```python
from build123d import *

# Parameters (mm, degrees)
SKETCH1_R           = 8
BOSS_EXTRUDE1_DEPTH = 16
FILLET1_R           = 2
FILLET2_R           = 2


with BuildPart() as part:
    # Sketch1 → Boss-Extrude1 (new body)
    with BuildSketch(Plane(origin=(0, 0, 0), x_dir=(1, 0, 0), z_dir=(0, 1, 0))):
        Polygon((5.636967427, -10.593611199), (11.992820129, -0.415048607), (6.355852702, 10.178562591), (-5.636967427, 10.593611199), (-11.992820129, 0.415048607), (-6.355852702, -10.178562591), align=None)
        with Locations(Location((0, 0, 0), (0, 0, 270))):
            Circle(SKETCH1_R, mode=Mode.SUBTRACT)
    extrude(amount=BOSS_EXTRUDE1_DEPTH)

    # Fillet1
    fillet1_edges = [part.edges().sort_by_distance(p)[0] for p in [
        (5.636967427, 8, 10.593611199),
    ]]
    fillet(fillet1_edges, radius=FILLET1_R)

    # Fillet2
    fillet2_edges = [part.edges().sort_by_distance(p)[0] for p in [
        (-6.355852702, 8, 10.178562591),
        (-11.992820129, 8, -0.415048607),
        (-5.636967427, 8, -10.593611199),
        (6.355852702, 8, -10.178562591),
        (11.992820129, 8, 0.415048607),
    ]]
    fillet(fillet2_edges, radius=FILLET2_R)


solid = part.part
```
Geometry check sheet. Reference: the model listing, model coordinates, mm. Give positions to 0.01 mm unless a question says otherwise; leave off trailing zeros. Order: outer loops, then holes, each group sorted by start corner. A loop starts at its lowest first (then second) coordinate and runs counter-clockwise, first axis right, second up.
1. Section check B-B, the plane z = 2.75. Enter the section's corners in (x, y), and give its area (3 significant figures).
2. Section check D-D, the plane z = -8.5. Enter the section's corners in (x, y), and give its area (3 significant figures).
3. Section check C-C, the plane x = 0. Enter the section's corners in (y, z).
4. Release check for a two-part mould opening along Z. For faces 1 (the face through (6.2, 8.11, -9.91)), 2 (the face through (8.78, 7.89, 5.56)), 3 (the face through (-7.81, 7.89, -1.73)) record: pulls with the +Z half, pulls with the -Z half, needs draft (parallel to the pull), parting line crosses it, or undercut.
5. Gauge pin test, flat ends, axial feed: pin 1 Ø1 at (x, z) = (-9, 3) entering from -Y; pin 2 Ø6 at (y, z) = (2, 7.5) entering from -X; pin 3 Ø4 at (x, z) = (0, -4) entering from -Y; pin 4 Ø5 at (x, y) = (-1, 3.5) entering from -Z. Record the tip position at first contact, or that the pin passes through.
6. Section check A-A, the plane y = 4.75. Enter the section's corners in (x, z), and give its area (3 significant figures).
7. Thickness scan on L1, parallel to X at y = 10.5, z = 0; L2, parallel to Z at x = 2, y = 2.75; L3, parallel to X at y = 11.75, z = 2. Record the ranges inside material, lowest first.
Values follow:
1. outline: (-10.31, 0) - (-7.51, 0) - (-7.51, 16) - (-10.31, 16) - close; (7.51, 0) - (10.53, 0) - (10.53, 16) - (7.51, 16) - close
1. area: 93.1 mm2
2. outline: (-6.94, 0) - (7.25, 0) - (7.25, 16) - (-6.94, 16) - close
2. area: 227 mm2
3. outline: (0, -10.4) - (16, -10.4) - (16, -8) - (0, -8) - close; (0, 8) - (16, 8) - (16, 10.4) - (0, 10.4) - close
4. face 1: pulls with the -Z half
4. face 2: pulls with the +Z half
4. face 3: undercut
5. pin 1: stops at y = 0
5. pin 2: stops at x = -9.38
5. pin 3: passes through
5. pin 4: stops at z = -10.52
6. outline: (-11.45, 0.6) arc R2 ccw to (-11.38, -1.39) - (-6.25, -9.61) arc R2 ccw to (-4.48, -10.55) - (5.2, -10.22) arc R2 ccw to (6.9, -9.16) - (11.45, -0.6) arc R2 ccw to (11.38, 1.39) - (6.25, 9.61) arc R2 ccw to (4.48, 10.55) - (-5.2, 10.22) arc R2 ccw to (-6.9, 9.16) - close; hole circle Ø16 at (0, 0)
6. area: 172 mm2
7. L1: x = -11.66 to -8, 8 to 11.66
7. L2: z = -10.33 to -7.75, 7.75 to 10.47
7. L3: x = -10.71 to -7.75, 7.75 to 11
